Part model, mm, in its own coordinate system. A direction names the side the tool comes from. Give positions to 0.01 mm unless a question says otherwise; leave off trailing zeros. Write each loop counter-clockwise with the first axis right and the second up, starting at its lowest first coordinate (ties: lowest second). Pieces come first, ordered by that corner, then holes. Notation, with made-up numbers: (19.25, 78.5) - (50.25, 78.5) arc R13 cw to (50.25, 82.5) - close; hole circle Ø7 at (42, 12.25). An arc over 180 degrees is marked (long way). Answer in a Markdown table with one row per item. Add a question column.
1. Band-saw the part on D-D on y = 2.5. Write the cut outline in (x, z), plus the area to 3 significant figures.
2. Band-saw the part on C-C on z = 16.25. Write the cut outline in (x, y).
3. Probe line 1 along Z through (x, y) = (-1.75, -2.25); line 2 along X through (y, z) = (-0.25, 15.25); line 3 along Y through (x, z) = (2.25, 1.5). List the from-to ranges inside material, lowest first.
4. Band-saw the part on B-B on x = -2. Write the cut outline in (y, z), plus the area to 3 significant figures.
5. Drop flat-ended pins along their axis: pin 1 Ø1.5 at (x, z) = (-2.5, 12.5) entering from -Y; pin 2 Ø3 at (x, z) = (-0.5, 9) entering from +Y; pin 3 Ø2 at (x, y) = (-3, 0) entering from +Z. Give the stop position or say it passes through.
6. Band-saw the part on A-A on z = 9.75. Write the cut outline in (x, y).
7. Which spindle directions (+Z, -Z, +X, -X, +Y, -Y) get a long thin tool onto all of the face, cutting with end or side? Do faces 1 (the flat face through (-1, -3, 8)), 2 (the flat face through (1.8, 3, 9.2)), 3 (the cylindrical face through (-3, 0, 11)). Say none if no direction does.
```python
from build123d import *

# Parameters (mm, degrees)
SKETCH1_R           = 3
BOSS_EXTRUDE1_DEPTH = 8
BOSS_EXTRUDE2_DEPTH = 2.5
SKETCH3_R           = 3
BOSS_EXTRUDE3_DEPTH = 2
SKETCH4_R           = 0.4
BOSS_EXTRUDE4_DEPTH = 10


with BuildPart() as part:
    # Sketch1 → Boss-Extrude1 (new body)
    with BuildSketch(Plane.XY):
        Circle(SKETCH1_R)
    extrude(amount=BOSS_EXTRUDE1_DEPTH)

    # Sketch2 → Boss-Extrude2 (add)
    with BuildSketch(Plane.XY.offset(8)):
        Polygon((0, 4.041451884), (-3.5, 2.020725942), (-3.5, -2.020725942), (0, -4.041451884), (3.5, -2.020725942), (3.5, 2.020725942), align=None)
    extrude(amount=BOSS_EXTRUDE2_DEPTH)

    # Sketch3 → Boss-Extrude3 (add)
    with BuildSketch(Plane.XY.offset(10.5)):
        Circle(SKETCH3_R)
    extrude(amount=BOSS_EXTRUDE3_DEPTH)

    # Sketch4 → Boss-Extrude4 (add)
    with BuildSketch(Plane.XY.offset(12.5)):
        with Locations((0.5, 0)):
            Circle(SKETCH4_R)
        with Locations((-0.5, 0)):
            Circle(SKETCH4_R)
    extrude(amount=BOSS_EXTRUDE4_DEPTH)


solid = part.part
```
Values:
| question | item | result |
|---|---|---|
| 1 | outline | (-2.67, 8) - (-1.66, 8) - (-1.66, 0) - (1.66, 0) - (1.66, 8) - (2.67, 8) - (2.67, 10.5) - (1.66, 10.5) - (1.66, 12.5) - (-1.66, 12.5) - (-1.66, 10.5) - (-2.67, 10.5) - close |
| 1 | area | 46.5 mm² |
| 2 | outline | circle Ø0.8 at (-0.5, 0); circle Ø0.8 at (0.5, 0) |
| 3 | line 1 | z = 0 to 12.5 |
| 3 | line 2 | x = -0.81 to -0.19, 0.19 to 0.81 |
| 3 | line 3 | y = -1.98 to 1.98 |
| 4 | outline | (-2.89, 8) - (-2.24, 8) - (-2.24, 0) - (2.24, 0) - (2.24, 8) - (2.89, 8) - (2.89, 10.5) - (2.24, 10.5) - (2.24, 12.5) - (-2.24, 12.5) - (-2.24, 10.5) - (-2.89, 10.5) - close |
| 4 | area | 59.2 mm² |
| 5 | pin 1 | stops at y = -2.44 |
| 5 | pin 2 | stops at y = 4.04 |
| 5 | pin 3 | stops at z = 12.5 |
| 6 | outline | (-3.5, -2.02) - (0, -4.04) - (3.5, -2.02) - (3.5, 2.02) - (0, 4.04) - (-3.5, 2.02) - close |
| 7 | face 1 | -Z |
| 7 | face 2 | +Z, -Z, +X, +Y |
| 7 | face 3 | +Z |
